Here's how the part is built. I have some questions about the finished solid (model axes, mm). A direction names the side the tool comes from. Give positions to 0.01 mm unless a question says otherwise; leave off trailing zeros. Order: outer loops, then holes, each group sorted by start corner. A loop starts at its lowest first (then second) coordinate and runs counter-clockwise, first axis right, second up.
from build123d import *

# Parameters (mm, degrees)
SKETCH1_R               = 6
BOSS_EXTRUDE1_DEPTH     = 10
BOSS_EXTRUDE2_DEPTH     = 10
FILLET1_R               = 3
CUT_EXTRUDE1_DEPTH      = 128.867118525
CUT_EXTRUDE1_DEPTH_BACK = 10
SKETCH3_R               = 11


with BuildPart() as part:
    # Sketch1 → Boss-Extrude1 (new body)
    with BuildSketch(Plane.XY):
        Polygon((-65, 45), (-55, 55), (55, 55), (65, 45), (65, -45), (55, -55), (-55, -55), (-65, -45), align=None)
        with Locations((16.378850905, 39.542043991)):
            Circle(SKETCH1_R, mode=Mode.SUBTRACT)
        with Locations((39.542043991, 16.378850905)):
            Circle(SKETCH1_R, mode=Mode.SUBTRACT)
        with Locations((39.542043991, -16.378850905)):
            Circle(SKETCH1_R, mode=Mode.SUBTRACT)
        with Locations((16.378850905, -39.542043991)):
            Circle(SKETCH1_R, mode=Mode.SUBTRACT)
        with Locations((-16.378850905, -39.542043991)):
            Circle(SKETCH1_R, mode=Mode.SUBTRACT)
        with Locations((-39.542043991, -16.378850905)):
            Circle(SKETCH1_R, mode=Mode.SUBTRACT)
        with Locations((-39.542043991, 16.378850905)):
            Circle(SKETCH1_R, mode=Mode.SUBTRACT)
        with Locations((-16.378850905, 39.542043991)):
            Circle(SKETCH1_R, mode=Mode.SUBTRACT)
        with BuildLine():
            Line((5.447198752, 40.634715337), (-5.447198752, 40.634715337))
            ThreePointArc((-5.447198752, 40.634715337), (-6.861412314, 40.0489289), (-7.447198752, 38.634715337))
            Line((-7.447198752, 38.634715337), (-7.447198752, 15.245017914))
            ThreePointArc((-7.447198752, 15.245017914), (-6.861412314, 13.830804352), (-5.447198752, 13.245017914))
            Line((-5.447198752, 13.245017914), (5.447198752, 13.245017914))
            ThreePointArc((5.447198752, 13.245017914), (6.861412314, 13.830804352), (7.447198752, 15.245017914))
            Line((7.447198752, 15.245017914), (7.447198752, 38.634715337))
            ThreePointArc((7.447198752, 38.634715337), (6.861412314, 40.0489289), (5.447198752, 40.634715337))
        make_face(mode=Mode.SUBTRACT)
        with BuildLine():
            Line((15.245017914, -7.447198752), (38.634715337, -7.447198752))
            ThreePointArc((38.634715337, -7.447198752), (40.0489289, -6.861412314), (40.634715337, -5.447198752))
            Line((40.634715337, -5.447198752), (40.634715337, 5.447198752))
            ThreePointArc((40.634715337, 5.447198752), (40.0489289, 6.861412314), (38.634715337, 7.447198752))
            Line((38.634715337, 7.447198752), (15.245017914, 7.447198752))
            ThreePointArc((15.245017914, 7.447198752), (13.830804352, 6.861412314), (13.245017914, 5.447198752))
            Line((13.245017914, 5.447198752), (13.245017914, -5.447198752))
            ThreePointArc((13.245017914, -5.447198752), (13.830804352, -6.861412314), (15.245017914, -7.447198752))
        make_face(mode=Mode.SUBTRACT)
        with BuildLine():
            Line((-7.447198752, -15.245017914), (-7.447198752, -38.634715337))
            ThreePointArc((-7.447198752, -38.634715337), (-6.861412314, -40.0489289), (-5.447198752, -40.634715337))
            Line((-5.447198752, -40.634715337), (5.447198752, -40.634715337))
            ThreePointArc((5.447198752, -40.634715337), (6.861412314, -40.0489289), (7.447198752, -38.634715337))
            Line((7.447198752, -38.634715337), (7.447198752, -15.245017914))
            ThreePointArc((7.447198752, -15.245017914), (6.861412314, -13.830804352), (5.447198752, -13.245017914))
            Line((5.447198752, -13.245017914), (-5.447198752, -13.245017914))
            ThreePointArc((-5.447198752, -13.245017914), (-6.861412314, -13.830804352), (-7.447198752, -15.245017914))
        make_face(mode=Mode.SUBTRACT)
        with BuildLine():
            Line((-15.245017914, 7.447198752), (-38.634715337, 7.447198752))
            ThreePointArc((-38.634715337, 7.447198752), (-40.0489289, 6.861412314), (-40.634715337, 5.447198752))
            Line((-40.634715337, 5.447198752), (-40.634715337, -5.447198752))
            ThreePointArc((-40.634715337, -5.447198752), (-40.0489289, -6.861412314), (-38.634715337, -7.447198752))
            Line((-38.634715337, -7.447198752), (-15.245017914, -7.447198752))
            ThreePointArc((-15.245017914, -7.447198752), (-13.830804352, -6.861412314), (-13.245017914, -5.447198752))
            Line((-13.245017914, -5.447198752), (-13.245017914, 5.447198752))
            ThreePointArc((-13.245017914, 5.447198752), (-13.830804352, 6.861412314), (-15.245017914, 7.447198752))
        make_face(mode=Mode.SUBTRACT)
    extrude(amount=BOSS_EXTRUDE1_DEPTH)

    # Sketch2 → Boss-Extrude2 (add)
    with BuildSketch(Plane.XY):
        Polygon((-112, 25), (-65, 25), (-65, -25), (-112, -25), (-115, -22), (-115, 22), align=None)
        Polygon((115, -22), (112, -25), (65, -25), (65, 25), (112, 25), (115, 22), align=None)
    extrude(amount=BOSS_EXTRUDE2_DEPTH)

    # Fillet1
    fillet1_edges = [part.edges().sort_by_distance(p)[0] for p in [
        (-65, 25, 5),
        (-65, -25, 5),
    ]]
    fillet(fillet1_edges, radius=FILLET1_R)

    # Sketch3 → Cut-Extrude1 (cut, two sides: drawn at the far end of the back side and taken through both)
    with BuildSketch(Plane.XY.offset(10).offset(-CUT_EXTRUDE1_DEPTH_BACK)):
        with Locations(Location((0, 0, 0), (0, 0, 180))):
            Circle(SKETCH3_R)
    extrude(amount=CUT_EXTRUDE1_DEPTH + CUT_EXTRUDE1_DEPTH_BACK, mode=Mode.SUBTRACT)


solid = part.part
Q1. I'm going to push flat-ended pins straight in: P1, Ø5, axis at x = 58, z = 1.5, coming from the -Y side; P2, Ø3, axis at x = -84, z = 4.5, coming from the +Y side; P3, Ø3, axis at x = -97.5, z = 3.5, coming from the -Y side. Where does each tip first touch, or does it pass through?
Filled sheet:
P1: stops at y = -54.5
P2: stops at y = 25
P3: stops at y = -25
Q2. If we section it at D-D on y = 48.5: List the corners of the cut face in (x, z) for me.
Filled sheet:
outline: (-61.5, 0) - (61.5, 0) - (61.5, 10) - (-61.5, 10) - close
Q3. If we section it at A-A on y = 0: List the corners of the cut face in (x, z) for me, plus the area to 3 significant figures.
Filled sheet:
outline: (-115, 0) - (-40.63, 0) - (-40.63, 10) - (-115, 10) - close; (-13.25, 0) - (-11, 0) - (-11, 10) - (-13.25, 10) - close; (11, 0) - (13.25, 0) - (13.25, 10) - (11, 10) - close; (40.63, 0) - (115, 0) - (115, 10) - (40.63, 10) - close
area: 1,530 mm2
Q4. If we section it at B-B on x = 0: List the corners of the cut face in (y, z) for me.
Filled sheet:
outline: (-55, 0) - (-40.63, 0) - (-40.63, 10) - (-55, 10) - close; (-13.25, 0) - (-11, 0) - (-11, 10) - (-13.25, 10) - close; (11, 0) - (13.25, 0) - (13.25, 10) - (11, 10) - close; (40.63, 0) - (55, 0) - (55, 10) - (40.63, 10) - close
Q5. I need wall thicknesses on L1, parallel to X at y = 5, z = 4.75; L2, parallel to X at y = 19, z = 3; L3, parallel to Y at x = -41.5, z = 8.75. Which ranges of each line are inside material? Lowest first, please.
Filled sheet:
L1: x = -115 to -40.63, -13.25 to -9.8, 9.8 to 13.25, 40.63 to 115
L2: x = -115 to -44.94, -34.14 to -7.45, 7.45 to 34.14, 44.94 to 115
L3: y = -55 to -22.05, -10.71 to 10.71, 22.05 to 55
Q6. Thinking about a two-plate mould opening in X: for faces 1 (the face through (2, -11, 0)), 2 (the face through (65, 35, 5)), 3 (the face through (0, 13.245, 5)), which applies, released by +X, released by -X, zero draft, split by the parting line, or undercut?
Filled sheet:
face 1: zero draft
face 2: released by +X
face 3: undercut
Q7. For faces 4 (the face through (115, 0, 5)), 5 (the face through (0, -40.635, 5)), which set-ups out of +Z, -Z, +X, -X, +Y, -Y let a thin tool reach every point of the face, with its end or its side?
Filled sheet:
face 4: +Z, -Z, +X, +Y, -Y
face 5: +Z, -Z
Q8. If we section it at C-C on x = -72: List the corners of the cut face in (y, z) for me.
Filled sheet:
outline: (-25, 0) - (25, 0) - (25, 10) - (-25, 10) - close
